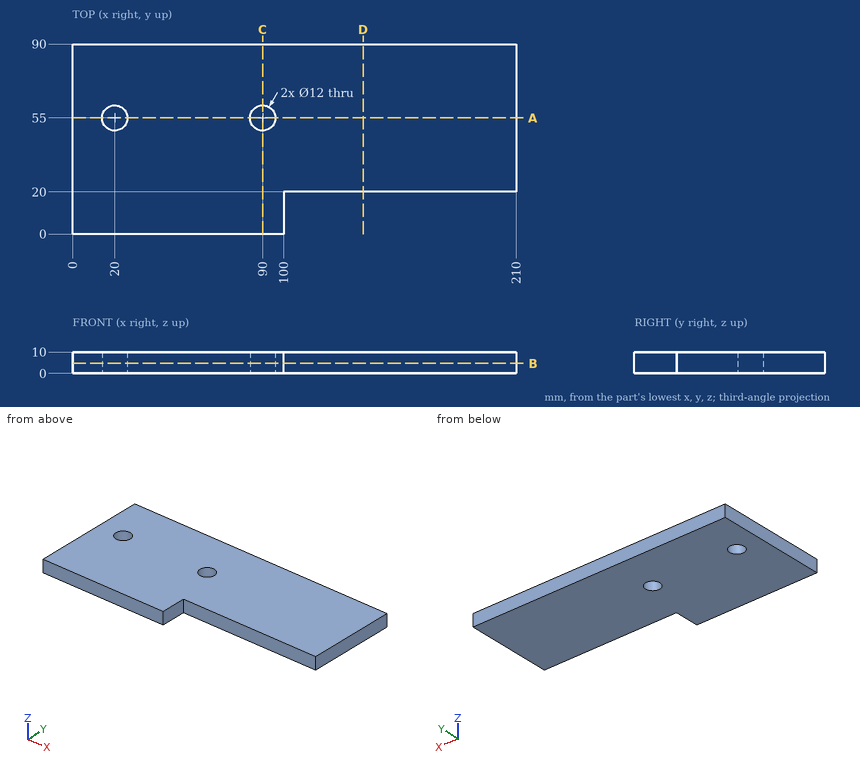
Here's the drawing with two shaded views (mm, measured from the low corner). I have some questions. Coordinates: 2 decimals unless noted, no trailing zeros. Order: outer loops, then holes, each group sorted by start corner. A loop starts at its lowest first (then second) coordinate and runs counter-clockwise, first axis right, second up. Notation, with made-up numbers: (9, -39.5) - (25, -39.5) arc R9 ccw to (25, -27.5) - close; hole circle Ø1 at (-11, 19.5). An arc over 180 degrees is marked (long way). Answer in a Markdown table with one row per item. Add a question column.
(1) Will these pins go through, and if not, where does the flat tip stop? pin 1 (5 mm diameter, centred on x = 145, z = 2, fed in from -Y); pin 2 (5 mm diameter, centred on y = 8.5, z = 6, fed in from +X).
(2) If we section it at B-B, the plane z = 4.75: Please give me the cut outline in (x, y), then the cut area to 3 significant figures.
(3) If we section it at D-D, the plane x = 137.5: Please give me the cut outline in (y, z).
(4) If we section it at A-A, the plane y = 55: Please give me the cut outline in (x, z), then the cut area to 3 significant figures.
(5) If we section it at C-C, the plane x = 90: Please give me the cut outline in (y, z), then the cut area to 3 significant figures.
(6) I need wall thicknesses on L1, parallel to X at y = 54.5, z = 7; L2, parallel to Y at x = 90, z = 6.75; L3, parallel to Y at x = 156, z = 3.5. Which ranges of each line are inside material? Lowest first, please.
Results are:
| question | item | result |
|---|---|---|
| 1 | pin 1 | stops at y = 20 |
| 1 | pin 2 | stops at x = 100 |
| 2 | outline | (0, 0) - (100, 0) - (100, 20) - (210, 20) - (210, 90) - (0, 90) - close; hole circle Ø12 at (20, 55); hole circle Ø12 at (90, 55) |
| 2 | area | 16,500 mm2 |
| 3 | outline | (20, 0) - (90, 0) - (90, 10) - (20, 10) - close |
| 4 | outline | (0, 0) - (14, 0) - (14, 10) - (0, 10) - close; (26, 0) - (84, 0) - (84, 10) - (26, 10) - close; (96, 0) - (210, 0) - (210, 10) - (96, 10) - close |
| 4 | area | 1,860 mm2 |
| 5 | outline | (0, 0) - (49, 0) - (49, 10) - (0, 10) - close; (61, 0) - (90, 0) - (90, 10) - (61, 10) - close |
| 5 | area | 780 mm2 |
| 6 | L1 | x = 0 to 14.02, 25.98 to 84.02, 95.98 to 210 |
| 6 | L2 | y = 0 to 49, 61 to 90 |
| 6 | L3 | y = 20 to 90 |
